from build123d import *

# Parameters (mm, degrees)
SKETCH1_R           = 35
BOSS_EXTRUDE1_DEPTH = 20
CHAMFER1_SIZE       = 5


with BuildPart() as part:
    # Sketch1 → Boss-Extrude1 (new body)
    with BuildSketch(Plane.XY):
        with BuildLine():
            ThreePointArc((72.887397787, -202.60557658), (27.017010086, -221.097976732), (4.818924287, -265.294201888))
            ThreePointArc((4.818924287, -265.294201888), (-64.294796067, -327.998176898), (-134.306386999, -266.298323103))
            ThreePointArc((-134.306386999, -266.298323103), (-144.622358434, -212.04763629), (-162.31184025, -159.734745723))
            ThreePointArc((-162.31184025, -159.734745723), (-154.669991707, 126.763312998), (64.446169212, 311.5))
            ThreePointArc((64.446169212, 311.5), (125.230637191, 300.548967821), (153.683278213, 245.729957687))
            ThreePointArc((153.683278213, 245.729957687), (167.70153078, 200.795951222), (203.480405215, 170.210848864))
            ThreePointArc((203.480405215, 170.210848864), (207.986601411, 166.133457037), (209.3, 160.2))
            Line((209.3, 160.2), (16.2, 177.8))
            Line((16.2, 177.8), (14.744884523, 161.829658531))
            ThreePointArc((14.744884523, 161.829658531), (-162.499999947, -0.00413168), (14.753113776, -161.828908523))
            Line((14.753113776, -161.828908523), (16.2, -177.7))
            Line((16.2, -177.7), (102.1, -169.9))
            ThreePointArc((102.1, -169.9), (94.597243609, -192.597670349), (72.887397787, -202.60557658))
        make_face()
        with Locations((-64.8, -258)):
            Circle(SKETCH1_R, mode=Mode.SUBTRACT)
        with Locations((83.7, 244.2)):
            Circle(SKETCH1_R, mode=Mode.SUBTRACT)
    extrude(amount=BOSS_EXTRUDE1_DEPTH)

    # Chamfer1
    chamfer1_edges = [part.edges().sort_by_distance(p)[0] for p in [
        (-162.499999947, -0.00413168, 0),
        (-162.499999947, -0.00413168, 20),
    ]]
    chamfer(chamfer1_edges, length=CHAMFER1_SIZE)


solid = part.part
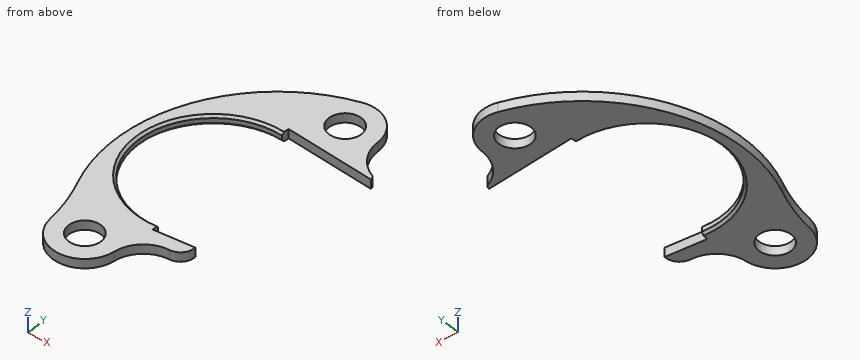
Verification items for the finished model (mm, model axes). Give positions to 0.01 mm unless a question says otherwise; leave off trailing zeros. Loops run counter-clockwise (first coordinate to the right, second up) from the corner with the lowest first, then second, coordinate; pieces in that order, holes last.
1) Sectioned sample at C-C, the plane y = -258. Enter the section's corners in (x, z).
2) Sectioned sample at B-B, the plane x = 83.7. Enter the section's corners in (y, z), then the cut area to 3 significant figures.
3) Depth check by flat-ended pin: pin 1 Ø4 at (x, z) = (146, 14.5) entering from +Y; pin 2 Ø10 at (x, z) = (146, 2.5) entering from +Y; pin 3 Ø3 at (x, z) = (-141.5, 8.5) entering from +Y. Enter the tip coordinate at first touch or a pass-through.
4) Thickness scan on line 1 along Y through (x, z) = (-53.5, 12); line 2 along Y through (x, z) = (-85.5, 11.5); line 3 along Y through (x, z) = (19.5, 10.5). Record the ranges inside material, lowest first.
5) Sectioned sample at D-D, the plane y = 0. Enter the section's corners in (x, z).
6) Sectioned sample at A-A, the plane z = 9. Enter the section's corners in (x, y), then the cut area to 3 significant figures.
Answers:
1. outline: (-135.39, 0) - (-99.8, 0) - (-99.8, 20) - (-135.39, 20) - close; (-29.8, 0) - (5.97, 0) - (5.97, 20) - (-29.8, 20) - close
2. outline: (-200.33, 0) - (-171.57, 0) - (-171.57, 20) - (-200.33, 20) - close; (171.65, 0) - (209.2, 0) - (209.2, 20) - (171.65, 20) - close; (279.2, 0) - (314.2, 0) - (314.2, 20) - (279.2, 20) - close
2. area: 2,030 mm2
3. pin 1: stops at y = 279.75
3. pin 2: stops at y = 284.41
3. pin 3: stops at y = 154.08
4. line 1: y = -327.08 to -291.13, -224.87 to -153.44, 153.44 to 251.79
4. line 2: y = -324.87 to -286.22, -229.78 to -138.19, 138.19 to 223.75
4. line 3: y = -229.21 to -177.4, 177.5 to 295.25
5. outline: (-188.39, 0) - (-167.5, 0) - (-162.5, 5) - (-162.5, 15) - (-167.5, 20) - (-188.39, 20) - close
6. outline: (-162.31, -159.73) arc R400 cw to (-134.31, -266.3) arc R70 ccw to (4.82, -265.29) arc R70 cw to (72.89, -202.61) arc R30 ccw to (102.1, -169.9) - (16.2, -177.7) - (14.75, -161.83) arc R162.5 cw (long way) to (14.74, 161.83) - (16.2, 177.8) - (209.3, 160.2) arc R10 ccw to (203.48, 170.21) arc R85 cw to (153.68, 245.73) arc R70 ccw to (64.45, 311.5) arc R350 ccw to start; hole circle Ø70 at (-64.8, -258); hole circle Ø70 at (83.7, 244.2)
6. area: 65,000 mm2
